The model under review builds one solid part; all positions refer to its coordinate system, in mm. Face numbers are marked on the shaded views. Give positions to 0.01 mm unless a question says otherwise; leave off trailing zeros. Loops run counter-clockwise (first coordinate to the right, second up) from the corner with the lowest first, then second, coordinate; pieces in that order, holes last. Notation, with made-up numbers: (62, 1.25) - (66, 1.25) arc R17 ccw to (66, 31.25) - close; hole circle Ø2 at (60, -33). An arc over 180 degrees is marked (long way). Return JSON: item names as keys, results as strings. Group by question number.
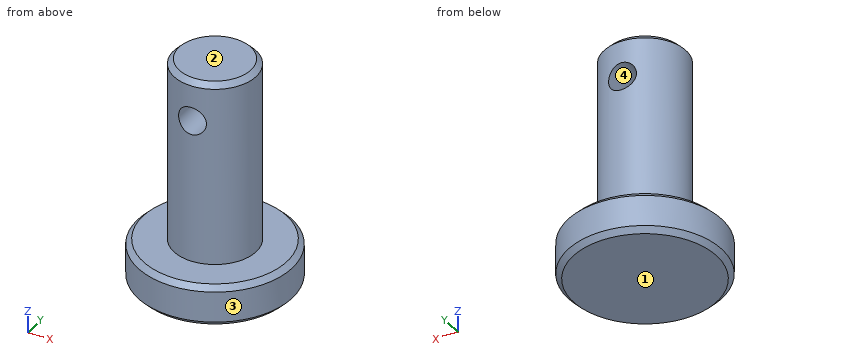
```python
from build123d import *

# Parameters (mm, degrees)
SKETCH1_R               = 4
BOSS_EXTRUDE1_DEPTH     = 18
SKETCH2_R               = 7.5
BOSS_EXTRUDE2_DEPTH     = 4
CUT_EXTRUDE1_DEPTH      = 21.892582416
CUT_EXTRUDE1_DEPTH_BACK = 21.892582416
SKETCH3_R               = 1.35
CHAMFER1_SIZE           = 0.5


with BuildPart() as part:
    # Sketch1 → Boss-Extrude1 (new body)
    with BuildSketch(Plane.XY):
        Circle(SKETCH1_R)
    extrude(amount=BOSS_EXTRUDE1_DEPTH)

    # Sketch2 → Boss-Extrude2 (add)
    with BuildSketch(Plane(origin=(0, 0, 0), x_dir=(-1, 0, 0), z_dir=(0, 0, -1))):
        Circle(SKETCH2_R)
    extrude(amount=BOSS_EXTRUDE2_DEPTH)

    # Sketch3 → Cut-Extrude1 (cut, two sides: drawn at the far end of the back side and taken through both)
    with BuildSketch(Plane(origin=(0, 0, 0), x_dir=(1, 0, 0), z_dir=(0, 1, 0)).offset(-CUT_EXTRUDE1_DEPTH_BACK)):
        with Locations(Location((0, -14, 0), (0, 0, 270))):
            Circle(SKETCH3_R)
    extrude(amount=CUT_EXTRUDE1_DEPTH + CUT_EXTRUDE1_DEPTH_BACK, mode=Mode.SUBTRACT)

    # Chamfer1
    chamfer1_edges = [part.edges().sort_by_distance(p)[0] for p in [
        (-4, 0, 18),
        (7.5, 0, 0),
        (7.5, 0, -4),
    ]]
    chamfer(chamfer1_edges, length=CHAMFER1_SIZE)


solid = part.part
```
1) To check wall thickness, follow line 1 (Z direction, x = 0, y = -2.5); line 2 (Z direction, x = 5, y = -4.75); line 3 (X direction, y = -2, z = 14). State the ranges of each line that lie inside material, in increasing order.
2) We need section D-D, the plane z = 0.75. Write out the cut boundary in (x, y), plus the area to 3 significant figures.
3) For pin 1 Ø4 at (y, z) = (-1, 10.5) entering from -X; pin 2 Ø4 at (y, z) = (5, 13) entering from +X; pin 3 Ø4.5 at (x, z) = (0, 14) entering from +Y, all flat-tipped, find the tip position at first contact; note any pin that passes through.
4) We need section C-C, the plane z = 15. Write out the cut boundary in (x, y), plus the area to 3 significant figures.
5) We need section A-A, the plane x = 0. Write out the cut boundary in (y, z), plus the area to 3 significant figures.
6) Draft analysis for pull direction Z (two halves, no side actions). For the marked faces 1, 2, 3 and 4, state which applies: +Z half, -Z half, draft (parallel to the pull), parting line (faces both ways), or undercut.
7) We need section B-B, the plane y = 0. Write out the cut boundary in (x, z), plus the area to 3 significant figures.
Findings:
{
 "1": {"line 1": "z = -4 to 12.65, 15.35 to 18", "line 2": "z = -4 to 0", "line 3": "x = -3.46 to -1.35, 1.35 to 3.46"},
 "2": {"outline": "circle Ø8 at (0, 0)", "area": "50.3 mm^2"},
 "3": {"pin 1": "stops at x = -4", "pin 2": "stops at x = 2.65", "pin 3": "stops at y = 4"},
 "4": {"outline": "(-0.91, -3.9) - (-0.91, 3.9) arc R4 ccw to start; (0.91, -3.9) arc R4 ccw to (0.91, 3.9) - close", "area": "35.9 mm^2"},
 "5": {"outline": "(-7.5, -3.5) - (-7, -4) - (7, -4) - (7.5, -3.5) - (7.5, -0.5) - (7, 0) - (4, 0) - (4, 12.65) - (-4, 12.65) - (-4, 0) - (-7, 0) - (-7.5, -0.5) - close; (-4, 15.35) - (4, 15.35) - (4, 17.5) - (3.5, 18) - (-3.5, 18) - (-4, 17.5) - close", "area": "182 mm^2"},
 "6": {"face 1": "-Z half", "face 2": "+Z half", "face 3": "draft", "face 4": "undercut"},
 "7": {"outline": "(-7.5, -3.5) - (-7, -4) - (7, -4) - (7.5, -3.5) - (7.5, -0.5) - (7, 0) - (4, 0) - (4, 17.5) - (3.5, 18) - (-3.5, 18) - (-4, 17.5) - (-4, 0) - (-7, 0) - (-7.5, -0.5) - close; hole circle Ø2.7 at (0, 14)", "area": "198 mm^2"}
}
